Geometry check sheet. Reference: the model listing, model coordinates, mm. A direction names the side the tool comes from. Round coordinates to 2 decimals unless told otherwise and drop trailing zeros. Order: outer loops, then holes, each group sorted by start corner. A loop starts at its lowest first (then second) coordinate and runs counter-clockwise, first axis right, second up.
```python
from build123d import *

# Parameters (mm, degrees)
L_ANGLE_PROFILE_SKETCH_W       = 150
L_ANGLE_PROFILE_SKETCH_H       = 10
L_ANGLE_PROFILE_SKETCH_W_2     = 10
L_ANGLE_PROFILE_SKETCH_H_2     = 100
L_ANGLE_BASE_DEPTH             = 43
UPRIGHT_TAB_AND_SLOT_CUT_DEPTH = 116
CLAMP_ARM_PROFILE_SKETCH_R     = 7.5
CLAMP_ARM_PROFILE_CUT_DEPTH    = 116


with BuildPart() as part:
    # L-Angle Profile Sketch → L-Angle Base (new, symmetric)
    with BuildSketch(Plane.XY):
        with Locations((-75, 5)):
            Rectangle(L_ANGLE_PROFILE_SKETCH_W, L_ANGLE_PROFILE_SKETCH_H)
        with Locations((5, 50)):
            Rectangle(L_ANGLE_PROFILE_SKETCH_W_2, L_ANGLE_PROFILE_SKETCH_H_2)
    extrude(amount=L_ANGLE_BASE_DEPTH, both=True)

    # Upright Tab and Slot Sketch → Upright Tab and Slot Cut (cut)
    with BuildSketch(Plane.ZY):
        with BuildLine():
            Line((7, 50), (7, 25))
            ThreePointArc((7, 25), (0, 18), (-7, 25))
            Line((-7, 25), (-7, 50))
            ThreePointArc((-7, 50), (0, 57), (7, 50))
        make_face()
        with BuildLine():
            Line((-25, 50), (-25, 10))
            Line((-25, 10), (-59.506944139, 10))
            Line((-59.506944139, 10), (-59.506944139, 107.254315339))
            Line((-59.506944139, 107.254315339), (43, 107.254315339))
            Line((43, 107.254315339), (43, 10))
            Line((43, 10), (25, 10))
            Line((25, 10), (25, 50))
            ThreePointArc((25, 50), (0, 75), (-25, 50))
        make_face()
    extrude(amount=-UPRIGHT_TAB_AND_SLOT_CUT_DEPTH, mode=Mode.SUBTRACT)

    # Clamp Arm Profile Sketch → Clamp Arm Profile Cut (cut)
    with BuildSketch(Plane(origin=(0, 10, 0), x_dir=(1, 0, 0), z_dir=(0, 1, 0))):
        with Locations(Location((-95, 0, 0), (0, 0, 180))):
            Circle(CLAMP_ARM_PROFILE_SKETCH_R)
        with BuildLine():
            Line((10, -25), (10, -43))
            Line((10, -43), (-150, -43))
            Line((-150, -43), (-150, 43))
            Line((-150, 43), (10, 43))
            Line((10, 43), (10, 25))
            Line((10, 25), (-17.151864589, 25))
            ThreePointArc((-17.151864589, 25), (-20.83176495, 25.701702665), (-23.995226133, 27.708333333))
            ThreePointArc((-23.995226133, 27.708333333), (-42.517796957, 37.256095308), (-63.29044546, 35.600057015))
            Line((-63.29044546, 35.600057015), (-57.34436202, 22.848639927))
            ThreePointArc((-57.34436202, 22.848639927), (-39.857161718, -21.751386889), (-62.782208742, 20.312930357))
            Line((-62.782208742, 20.312930357), (-68.728292182, 33.064347445))
            ThreePointArc((-68.728292182, 33.064347445), (-71.807070885, 31.119955968), (-74.685606061, 28.889805354))
            ThreePointArc((-74.685606061, 28.889805354), (-85.712027428, 21.739686255), (-98.220588235, 17.709540124))
            ThreePointArc((-98.220588235, 17.709540124), (-113, 0), (-98.220588235, -17.709540124))
            ThreePointArc((-98.220588235, -17.709540124), (-85.712027428, -21.739686255), (-74.685606061, -28.889805354))
            ThreePointArc((-74.685606061, -28.889805354), (-49.114550984, -37.989682547), (-23.995226133, -27.708333333))
            ThreePointArc((-23.995226133, -27.708333333), (-20.83176495, -25.701702665), (-17.151864589, -25))
            Line((-17.151864589, -25), (10, -25))
        make_face()
    extrude(amount=-CLAMP_ARM_PROFILE_CUT_DEPTH, mode=Mode.SUBTRACT)


solid = part.part
```
(1) Sectioned sample at D-D, the plane z = 22. Record the cut outline in (x, y), and give its area (3 significant figures).
Returned:
outline: (-85.17, 0) - (-59.59, 0) - (-59.59, 10) - (-85.17, 10) - close; (-40.41, 0) - (10, 0) - (10, 61.87) - (0, 61.87) - (0, 10) - (-40.41, 10) - close
area: 1,280 mm2
(2) Sectioned sample at A-A, the plane x = -50. Record the cut outline in (y, z).
Returned:
outline: (0, -38) - (10, -38) - (10, -24) - (0, -24) - close; (0, 24) - (10, 24) - (10, 38) - (0, 38) - close
(3) Set-up check for faces 4 (the flat face through (3, 20, -25)), 5 (the cylindrical face through (5, 57, 0)), 6 (the cylindrical face through (-38.948, 5.07, 21.304)), 7 (the flat face through (0, 42, 11)): record each of +Z, -Z, +X, -X, +Y, -Y from which the full face is reachable in a straight line by a thin tool's end or side.
Returned:
face 4: -Z, +X, +Y, -Y
face 5: +X, -X
face 6: +Y, -Y
face 7: +Z, -Z, -X, +Y
(4) Depth check by flat-ended pin: P1, Ø11, axis at x = 7, y = 43.5, coming from the -Z side; P2, Ø21.5, axis at x = 0.5, y = 35.5, coming from the +Z side; P3, Ø4, axis at y = 41.5, z = -4.5, coming from the +X side; P4, Ø4, axis at x = -91.5, z = -8.5, coming from the -Y side. Enter the tip coordinate at first touch or a pass-through.
Returned:
P1: stops at z = -25
P2: stops at z = 25
P3: passes through
P4: stops at y = 0
(5) Sectioned sample at B-B, the plane z = 0. Record the cut outline in (x, y).
Returned:
outline: (-113, 0) - (-102.5, 0) - (-102.5, 10) - (-113, 10) - close; (-87.5, 0) - (-74, 0) - (-74, 10) - (-87.5, 10) - close; (-26, 0) - (10, 0) - (10, 18) - (0, 18) - (0, 10) - (-26, 10) - close; (0, 57) - (10, 57) - (10, 75) - (0, 75) - close
(6) Draft check along Y on faces 1 (the flat face through (5, 38, 7)), 2 (the flat face through (-25, 0, 1)), 3 (the cylindrical face through (-50, 5, 38)). Enter one of: released by +Y, released by -Y, zero draft, split by the parting line, or undercut.
Returned:
face 1: undercut
face 2: released by -Y
face 3: zero draft
(7) Sectioned sample at C-C, the plane y = 20.5. Record the cut outline in (x, z).
Returned:
outline: (0, -25) - (10, -25) - (10, -5.36) - (0, -5.36) - close; (0, 5.36) - (10, 5.36) - (10, 25) - (0, 25) - close
(8) Material ranges on line 1 (Z direction, x = -50, y = 5.5); line 2 (Y direction, x = -41.5, z = 32.5), recorded low to high.
Returned:
line 1: z = -38 to -24, 24 to 38
line 2: y = 0 to 10
